Source: three-view drawing plus pictorial views. Frame: mm from the lowest corner of the part. A direction names the side the tool comes from. Give positions to 0.01 mm unless a question says otherwise; leave off trailing zeros. Order: outer loops, then holes, each group sorted by start corner. A loop starts at its lowest first (then second) coordinate and runs counter-clockwise, first axis right, second up. Notation, with made-up numbers: (83.5, 19) -> (99.5, 19) arc R31 ccw to (99.5, 47) -> close; hole circle Ø5 at (41, -29). An arc over 180 degrees is marked (long way). One line per question, with ' | ' between items.
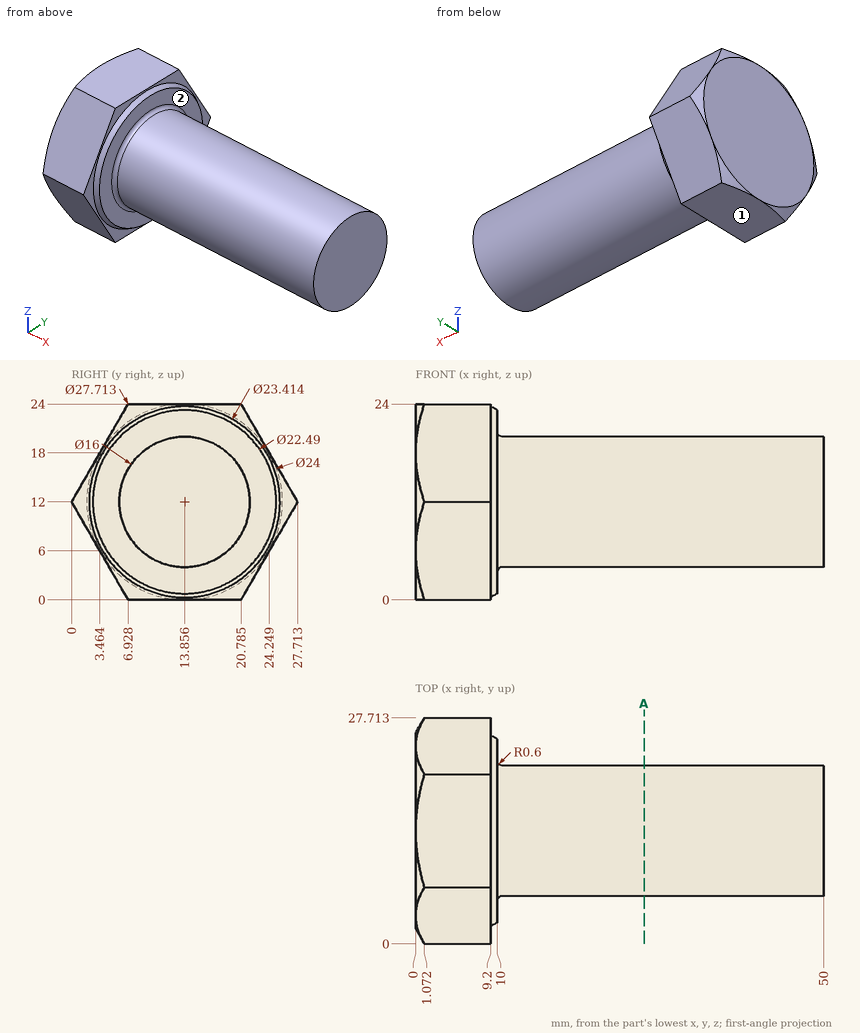
1) Contact query for flat-ended pins moving along their axis: pin 1 Ø5 at (y, z) = (23, 8) entering from +X; pin 2 Ø6 at (x, z) = (28, 4.5) entering from -Y; pin 3 Ø5 at (x, y) = (30, 8) entering from +Z; pin 4 Ø5 at (x, z) = (23.5, 13.5) entering from +Y. Output: stop coordinate, or through.
Check result:
pin 1: stops at x = 50 | pin 2: stops at y = 7.24 | pin 3: stops at z = 19.26 | pin 4: stops at y = 21.86
2) Section A-A on x = 28. Return loops of the section in (y, z), plus the area to 3 significant figures.
Check result:
outline: circle Ø16 at (13.86, 12) | area: 201 mm^2
3) Set-up query: the marked faces 1 and 2. Return all of +Z, -Z, +X, -X, +Y, -Y with unobstructed straight access to the full face (end or side cutting, diameter ignored); none if empty.
Check result:
face 1: -Z, +X, -X, +Y, -Y | face 2: +X
4) Material intervals for probe 1 along X at (y, z) = (23.75, 12.25); probe 2 along Y at (x, z) = (42, 13); probe 3 along X at (y, z) = (19.5, 2), sorted ascending. Write a range as from..to.
Check result:
probe 1: x = 0..10 | probe 2: y = 5.92..21.79 | probe 3: x = 0..9.59
